from build123d import *

# Parameters (mm, degrees)
SKETCH1_W           = 75
SKETCH1_H           = 75
BOSS_EXTRUDE1_DEPTH = 5
CUT_EXTRUDE1_DEPTH  = 5
SKETCH3_W           = 20
SKETCH3_H           = 40
CUT_EXTRUDE2_DEPTH  = 5
CUT_EXTRUDE3_REACH  = 55.268
SKETCH4_W           = 5
SKETCH4_H           = 14
SKETCH4_H_2         = 5
SKETCH4_H_3         = 10
CUT_EXTRUDE4_REACH  = 55.268
SKETCH5_W           = 5
SKETCH5_H           = 5
SKETCH5_H_2         = 14
SKETCH5_H_3         = 10
SKETCH7_W           = 65
SKETCH7_H           = 5
CUT_EXTRUDE5_DEPTH  = 10


with BuildPart() as part:
    # Sketch1 → Boss-Extrude1 (new body)
    with BuildSketch(Plane.XY):
        Rectangle(SKETCH1_W, SKETCH1_H)
    extrude(amount=BOSS_EXTRUDE1_DEPTH)

    # Sketch2 → Cut-Extrude1 (cut)
    with BuildSketch(Plane.XY.offset(5)):
        Polygon((-27.5, 37.5), (-37.5, 22.5), (-37.5, 37.5), align=None)
        Polygon((37.5, 37.5), (27.5, 37.5), (37.5, 22.5), align=None)
    extrude(amount=-CUT_EXTRUDE1_DEPTH, mode=Mode.SUBTRACT)

    # Sketch3 → Cut-Extrude2 (cut)
    with BuildSketch(Plane.XY.offset(5)):
        with Locations((-17.5, -17.5)):
            Rectangle(SKETCH3_W, SKETCH3_H)
    extrude(amount=-CUT_EXTRUDE2_DEPTH, mode=Mode.SUBTRACT)

    # Sketch4 → Cut-Extrude3 (cut, up to next)
    with BuildSketch(Plane.XY.offset(5), mode=Mode.PRIVATE) as cut_extrude3_sk1:
        with Locations((-35, -30.5)):
            Rectangle(SKETCH4_W, SKETCH4_H)
    cut_extrude3_tool1 = extrude(cut_extrude3_sk1.sketch, amount=-CUT_EXTRUDE3_REACH, mode=Mode.PRIVATE) & part.part
    # Sketch4 → Cut-Extrude3 (cut, up to next)
    with BuildSketch(Plane.XY.offset(5), mode=Mode.PRIVATE) as cut_extrude3_sk2:
        with Locations((-35, -16)):
            Rectangle(SKETCH4_W, SKETCH4_H_2)
    cut_extrude3_tool2 = extrude(cut_extrude3_sk2.sketch, amount=-CUT_EXTRUDE3_REACH, mode=Mode.PRIVATE) & part.part
    # Sketch4 → Cut-Extrude3 (cut, up to next)
    with BuildSketch(Plane.XY.offset(5), mode=Mode.PRIVATE) as cut_extrude3_sk3:
        with Locations((-35, -6)):
            Rectangle(SKETCH4_W, SKETCH4_H_2)
    cut_extrude3_tool3 = extrude(cut_extrude3_sk3.sketch, amount=-CUT_EXTRUDE3_REACH, mode=Mode.PRIVATE) & part.part
    # Sketch4 → Cut-Extrude3 (cut, up to next)
    with BuildSketch(Plane.XY.offset(5), mode=Mode.PRIVATE) as cut_extrude3_sk4:
        with Locations((-35, 6.5)):
            Rectangle(SKETCH4_W, SKETCH4_H_3)
    cut_extrude3_tool4 = extrude(cut_extrude3_sk4.sketch, amount=-CUT_EXTRUDE3_REACH, mode=Mode.PRIVATE) & part.part
    add(cut_extrude3_tool1.solids().sort_by_distance((-35, -30.5, 5))[0], mode=Mode.SUBTRACT)
    add(cut_extrude3_tool2.solids().sort_by_distance((-35, -16, 5))[0], mode=Mode.SUBTRACT)
    add(cut_extrude3_tool3.solids().sort_by_distance((-35, -6, 5))[0], mode=Mode.SUBTRACT)
    add(cut_extrude3_tool4.solids().sort_by_distance((-35, 6.5, 5))[0], mode=Mode.SUBTRACT)

    # Sketch5 → Cut-Extrude4 (cut, up to next)
    with BuildSketch(Plane.XY.offset(5), mode=Mode.PRIVATE) as cut_extrude4_sk1:
        with Locations((35, -16)):
            Rectangle(SKETCH5_W, SKETCH5_H)
    cut_extrude4_tool1 = extrude(cut_extrude4_sk1.sketch, amount=-CUT_EXTRUDE4_REACH, mode=Mode.PRIVATE) & part.part
    # Sketch5 → Cut-Extrude4 (cut, up to next)
    with BuildSketch(Plane.XY.offset(5), mode=Mode.PRIVATE) as cut_extrude4_sk2:
        with Locations((35, -6)):
            Rectangle(SKETCH5_W, SKETCH5_H)
    cut_extrude4_tool2 = extrude(cut_extrude4_sk2.sketch, amount=-CUT_EXTRUDE4_REACH, mode=Mode.PRIVATE) & part.part
    # Sketch5 → Cut-Extrude4 (cut, up to next)
    with BuildSketch(Plane.XY.offset(5), mode=Mode.PRIVATE) as cut_extrude4_sk3:
        with Locations((35, -30.5)):
            Rectangle(SKETCH5_W, SKETCH5_H_2)
    cut_extrude4_tool3 = extrude(cut_extrude4_sk3.sketch, amount=-CUT_EXTRUDE4_REACH, mode=Mode.PRIVATE) & part.part
    # Sketch5 → Cut-Extrude4 (cut, up to next)
    with BuildSketch(Plane.XY.offset(5), mode=Mode.PRIVATE) as cut_extrude4_sk4:
        with Locations((35, 6.5)):
            Rectangle(SKETCH5_W, SKETCH5_H_3)
    cut_extrude4_tool4 = extrude(cut_extrude4_sk4.sketch, amount=-CUT_EXTRUDE4_REACH, mode=Mode.PRIVATE) & part.part
    add(cut_extrude4_tool1.solids().sort_by_distance((35, -16, 5))[0], mode=Mode.SUBTRACT)
    add(cut_extrude4_tool2.solids().sort_by_distance((35, -6, 5))[0], mode=Mode.SUBTRACT)
    add(cut_extrude4_tool3.solids().sort_by_distance((35, -30.5, 5))[0], mode=Mode.SUBTRACT)
    add(cut_extrude4_tool4.solids().sort_by_distance((35, 6.5, 5))[0], mode=Mode.SUBTRACT)

    # Sketch7 → Cut-Extrude5 (cut)
    with BuildSketch(Plane.XY.offset(5)):
        with Locations((0, -35)):
            Rectangle(SKETCH7_W, SKETCH7_H)
    extrude(amount=-CUT_EXTRUDE5_DEPTH, mode=Mode.SUBTRACT)


solid = part.part
Input: part model. Units: mm. Frame: model coordinates. A direction names the side the tool comes from. Round coordinates to 2 decimals unless told otherwise and drop trailing zeros. Loops run counter-clockwise (first coordinate to the right, second up) from the corner with the lowest first, then second, coordinate; pieces in that order, holes last. Notation, with made-up numbers: M 50,-15 L 91,-15 A15 cw 91,13 Z; hole C 24,-26 d9. An arc over 180 degrees is marked long. Answer as CSV lines item,"result". Start each with the question number.
(1) Section A-A, the plane y = -0.5. Output: boundary loops of the cut face in (x, z).
(2) Section D-D, the plane x = -21. Output: boundary loops of the cut face in (y, z).
(3) Reachability of faces 1 (the flat face through (35, -8.5, 3)), 2 (the flat face through (12, -32.5, 3)), 3 (the flat face through (-35, -8.5, 3)) from +Z, -Z, +X, -X, +Y, -Y: full face, straight path, thin tool, end or side. Return the list, or none.
(4) First-contact query: pin 1 (2.5 mm diameter, centred on x = 35.5, z = 3.5, fed in from -Y); pin 2 (1.5 mm diameter, centred on y = 5, z = 1.5, fed in from +X); pin 3 (2.5 mm diameter, centred on y = -17, z = 3, fed in from -X). Flat tips, straight axial feed; report the tip coordinate or a pass-through.
(5) Draft query along Y for faces 4 (the flat face through (-18, 2.5, 3)), 5 (the flat face through (-32.5, 6, 3)), 6 (the flat face through (-35, -13.5, 3)), 7 (the flat face through (-37.5, -11, 2)). Return one class per face: released by +Y, released by -Y, zero draft, split by the parting line, or undercut.
(6) Section B-B, the plane y = -7.5. Output: boundary loops of the cut face in (x, z).
(7) Section C-C, the plane x = 31.5. Output: boundary loops of the cut face in (y, z).
(8) Line query: line 1 (X direction, y = -20.5, z = 2.65); line 2 (Y direction, x = 34, z = 3.2); line 3 (X direction, y = -14, z = 2). Output: solid intervals per line, ascending. Write a range as [from, to].
Values found:
1,outline,"M -37.5,0 L -27.5,0 L -27.5,5 L -37.5,5 Z; M -7.5,0 L 37.5,0 L 37.5,5 L -7.5,5 Z"
2,outline,"M 2.5,0 L 37.5,0 L 37.5,5 L 2.5,5 Z"
3,face 1,"+Z, -Z, +X"
3,face 2,"+Z, -Z, +X, -X, -Y"
3,face 3,"+Z, -Z, -X"
4,pin 1,"stops at y = -23.5"
4,pin 2,"stops at x = 32.5"
4,pin 3,"stops at x = -32.5"
5,face 4,"released by -Y"
5,face 5,"undercut"
5,face 6,"undercut"
5,face 7,"zero draft"
6,outline,"M -32.5,0 L -27.5,0 L -27.5,5 L -32.5,5 Z; M -7.5,0 L 32.5,0 L 32.5,5 L -7.5,5 Z"
7,outline,"M -32.5,0 L 31.5,0 L 31.5,5 L -32.5,5 Z"
8,line 1,"x = [-37.5, -27.5], [-7.5, 37.5]"
8,line 2,"y = [-23.5, -18.5], [-13.5, -8.5], [-3.5, 1.5], [11.5, 27.75]"
8,line 3,"x = [-32.5, -27.5], [-7.5, 32.5]"
